Read the model definition and answer for the solid it produces. Units are mm, in the model's axes. A direction names the side the tool comes from. Round coordinates to 2 decimals unless told otherwise and drop trailing zeros. Order: outer loops, then holes, each group sorted by start corner. A loop starts at its lowest first (then second) coordinate and runs counter-clockwise, first axis right, second up. Notation, with made-up numbers: (-14.75, 22) -> (34.25, 22) arc R21 cw to (34.25, 40) -> close; hole circle Ø5 at (16, 5). An arc over 180 degrees is marked (long way). Answer as a JSON object with one key per item and string values. Group by question number.
Item 1: Consider probe 1 along Z at (x, y) = (-0.85, -3); probe 2 along Z at (x, y) = (-0.55, 8); probe 3 along Z at (x, y) = (2, -1.25). Determine where each line is inside the solid, lowest interval first. Write a range as from..to.
Item 2: Section B-B, the plane x = 1 is taken. Write down the section's boundary in (y, z).
Item 3: Section D-D, the plane y = -8.25 is taken. Write down the section's boundary in (x, z), plus the area to 4 significant figures.
Item 4: For faces 4 (the flat face through (-2.25, 0, 3)), 5 (the flat face through (0, 1.099, 6)), 6 (the flat face through (0, 1, 0)), determine the directions among +Z, -Z, +X, -X, +Y, -Y from which every point of the face is accessible in a straight line to the end or side of a thin tool.
Item 5: The mould has two halves that part along Z. Classify faces 1 (the flat face through (0, 12.5, 2)), 2 (the flat face through (0, 7, 5)), 3 (the cylindrical face through (0.031, -3.595, 1.044)): pulls with the +Z half, pulls with the -Z half, needs draft (parallel to the pull), parting line crosses it, or undercut.
Item 6: Section C-C, the plane z = 1.5 is taken. Write down the section's boundary in (x, y), plus the area to 3 significant figures.
Item 7: Given P1, Ø1.3, axis at x = -0.5, y = 7.5, coming from the +Z side; P2, Ø1.3, axis at x = -1, y = 6.5, coming from the -Z side; P3, Ø1.2, axis at x = -0.5, z = 6, coming from the +Y side; P4, Ø1.2, axis at x = 0, z = -0.5, coming from the +Y side, each flat-ended and moving along its own axis, determine where each tip first touches the part or whether it passes through.
Item 8: Section A-A, the plane y = -3 is taken. Write down the section's boundary in (x, z), plus the area to 3 significant figures.
from build123d import *

# Parameters (mm, degrees)
SKETCH43_W          = 4.5
SKETCH43_H          = 25
BOSS_EXTRUDE1_DEPTH = 7.5
BOSS_EXTRUDE2_DEPTH = 4.5
SKETCH45_R          = 0.75
CUT_EXTRUDE1_DEPTH  = 16.256146302
SKETCH46_W          = 2.5
SKETCH46_H          = 11.400602873
CUT_EXTRUDE2_DEPTH  = 16.256146302


with BuildPart() as part:
    # Sketch43 → Boss-Extrude1 (new body)
    with BuildSketch(Plane.XY):
        Rectangle(SKETCH43_W, SKETCH43_H)
    extrude(amount=BOSS_EXTRUDE1_DEPTH)

    # Sketch44 → Boss-Extrude2 (add)
    with BuildSketch(Plane(origin=(2.25, 0, 0), x_dir=(0, 0, -1), z_dir=(1, 0, 0))):
        Polygon((0, -12.5), (0.5, -12.5), (1.5, -11), (0, -11), align=None)
    extrude(amount=-BOSS_EXTRUDE2_DEPTH)

    # Sketch45 → Cut-Extrude1 (cut, through all)
    with BuildSketch(Plane(origin=(2.25, 0, 0), x_dir=(0, 0, -1), z_dir=(1, 0, 0))):
        with Locations(Location((-1.5, -3, 0), (0, 0, 90))):
            Circle(SKETCH45_R)
    extrude(amount=-CUT_EXTRUDE1_DEPTH, mode=Mode.SUBTRACT)

    # Sketch46 → Cut-Extrude2 (cut, through all)
    with BuildSketch(Plane.ZY.offset(2.25)):
        with Locations((6.25, 6.799698563)):
            Rectangle(SKETCH46_W, SKETCH46_H)
    extrude(amount=-CUT_EXTRUDE2_DEPTH, mode=Mode.SUBTRACT)


solid = part.part
Values found:
{
 "1": {"probe 1": "0..0.75, 2.25..7.5", "probe 2": "0..5", "probe 3": "0..7.5"},
 "2": {"outline": "(-12.5, -0.5) -> (-11, -1.5) -> (-11, 0) -> (12.5, 0) -> (12.5, 5) -> (1.1, 5) -> (1.1, 7.5) -> (-12.5, 7.5) -> close; hole circle Ø1.5 at (-3, 1.5)"},
 "3": {"outline": "(-2.25, 0) -> (2.25, 0) -> (2.25, 7.5) -> (-2.25, 7.5) -> close", "area": "33.75 mm2"},
 "4": {"face 4": "+Z, -Z, -X, +Y, -Y", "face 5": "+Z, +X, -X, +Y", "face 6": "-Z, +X, -X, +Y"},
 "5": {"face 1": "needs draft", "face 2": "pulls with the +Z half", "face 3": "undercut"},
 "6": {"outline": "(-2.25, -12.5) -> (2.25, -12.5) -> (2.25, -3.75) -> (-2.25, -3.75) -> close; (-2.25, -2.25) -> (2.25, -2.25) -> (2.25, 12.5) -> (-2.25, 12.5) -> close", "area": "106 mm2"},
 "7": {"P1": "z = 5", "P2": "z = 0", "P3": "y = 1.1", "P4": "y = 12.5"},
 "8": {"outline": "(-2.25, 0) -> (2.25, 0) -> (2.25, 0.75) -> (-2.25, 0.75) -> close; (-2.25, 2.25) -> (2.25, 2.25) -> (2.25, 7.5) -> (-2.25, 7.5) -> close", "area": "27.0 mm2"}
}
